Geometry: final body of the model. Coordinates: model frame, mm. A direction names the side the tool comes from. Round coordinates to 2 decimals unless told otherwise and drop trailing zeros. Loops run counter-clockwise (first coordinate to the right, second up) from the corner with the lowest first, then second, coordinate; pieces in that order, holes last. Notation, with made-up numbers: (-32.5, 17) - (15.5, 17) arc R21 cw to (15.5, 48) - close; hole circle Ø10 at (-3.75, 84). An arc over 180 degrees is marked (long way). Return JSON: item names as keys, results as strings. Group by question number.
1. Section A-A on z = 31.5. Return loops of the section in (x, y).
2. Set-up query: faces 1 (the face through (0, -4, 200)), 2 (the face through (-0.74, -3.32, 10.01)). Return all of +Z, -Z, +X, -X, +Y, -Y with unobstructed straight access to the full face (end or side cutting, diameter ignored); none if empty.
3. Draft query along X for faces 3 (the face through (0.74, -3.32, 189.99)), 4 (the face through (-2.17, -9.76, 98.61)), 5 (the face through (0, -4, 0)). Return one class per face: +X half, -X half, draft (parallel to the pull), parting line (faces both ways), or undercut.
4. First-contact query: pin 1 Ø6 at (x, y) = (-5.5, 4) entering from -Z; pin 2 Ø2 at (x, z) = (2, 158.5) entering from +Y; pin 3 Ø5.5 at (x, y) = (0, 0) entering from +Z; pin 4 Ø1 at (y, z) = (7, 90) entering from +X. Flat tips, straight axial feed; report the tip coordinate or a pass-through.
5. Material intervals for probe 1 along Y at (x, z) = (0, 12); probe 2 along Z at (x, y) = (6.75, 6); probe 3 along Y at (x, z) = (0.5, 113.5), sorted ascending.
from build123d import *

# Parameters (mm, degrees)
SKETCH_1_R             = 10
EXTRUDE_1_DEPTH        = 200
HOLE_WIZARD_M8_1_D     = 6.8
HOLE_WIZARD_M8_1_DEPTH = 19.75
HOLE_WIZARD_M8_1_TIP   = 2.042926105
HOLE_WIZARD_M8_2_D     = 6.8
HOLE_WIZARD_M8_2_DEPTH = 19.75
HOLE_WIZARD_M8_2_TIP   = 2.042926105
CHAMFER_1_SIZE         = 1


with BuildPart() as part:
    # 草图1 → 凸台-拉伸1 (new body)
    with BuildSketch(Plane.XY):
        Circle(SKETCH_1_R)
    extrude(amount=EXTRUDE_1_DEPTH)

    # M8 螺纹孔1
    with Locations(Plane(origin=(0, 0, 0), x_dir=(-1, 0, 0), z_dir=(0, 0, -1))):
        with Locations((0, 0)):
            Hole(HOLE_WIZARD_M8_1_D / 2, depth=HOLE_WIZARD_M8_1_DEPTH)
            with Locations((0, 0, -(HOLE_WIZARD_M8_1_DEPTH + HOLE_WIZARD_M8_1_TIP / 2))):  # 118° drill point
                Cone(0, HOLE_WIZARD_M8_1_D / 2, HOLE_WIZARD_M8_1_TIP, mode=Mode.SUBTRACT)

    # M8 螺纹孔2
    with Locations(Plane.XY.offset(200)):
        with Locations((0, 0)):
            Hole(HOLE_WIZARD_M8_2_D / 2, depth=HOLE_WIZARD_M8_2_DEPTH)
            with Locations((0, 0, -(HOLE_WIZARD_M8_2_DEPTH + HOLE_WIZARD_M8_2_TIP / 2))):  # 118° drill point
                Cone(0, HOLE_WIZARD_M8_2_D / 2, HOLE_WIZARD_M8_2_TIP, mode=Mode.SUBTRACT)

    # 倒角1
    chamfer_1_edges = [part.edges().sort_by_distance(p)[0] for p in [
        (-10, 0, 0),
        (-10, 0, 200),
    ]]
    chamfer(chamfer_1_edges, length=CHAMFER_1_SIZE)


solid = part.part
Taken from the geometry:
{
 "1": {"outline": "circle Ø20 at (0, 0)"},
 "2": {"face 1": "+Z, +X, -X, +Y, -Y", "face 2": "-Z"},
 "3": {"face 3": "undercut", "face 4": "parting line", "face 5": "draft"},
 "4": {"pin 1": "z = 0", "pin 2": "y = 9.95", "pin 3": "z = 179.86", "pin 4": "x = 7.6"},
 "5": {"probe 1": "-10 to -3.4, 3.4 to 10", "probe 2": "0.03 to 199.97", "probe 3": "-9.99 to 9.99"}
}
